Verification items for the finished model (mm, model axes). Face numbers are marked on the shaded views. A direction names the side the tool comes from. Coordinates: 2 decimals unless noted, no trailing zeros. Order: outer loops, then holes, each group sorted by start corner. A loop starts at its lowest first (then second) coordinate and runs counter-clockwise, first axis right, second up. Notation, with made-up numbers: M 46,51.25 L 94,51.25 A21 cw 94,79.25 Z; hole C -4.5,40.25 d3. An arc over 180 degrees is marked long. Return JSON: item names as keys, results as strings. Group by question number.
Q1. Go/stop test with flat-tipped pins: pin 1 Ø5.5 at (x, y) = (-2.5, 38) entering from +Z; pin 2 Ø5.5 at (x, y) = (0, 16) entering from -Z (3 decimals); pin 3 Ø5.5 at (x, y) = (1.5, 18) entering from +Z; pin 4 Ø1 at (x, y) = (-1.5, 4.5) entering from -Z. Record where each tip stops, or that it passes through.
Q2. Section check B-B, the plane z = 17. Enter the section's corners in (x, y).
Q3. Section check D-D, the plane y = -0.5. Enter the section's corners in (x, z), then the cut area to 3 significant figures.
Q4. Section check A-A, the plane y = 36. Enter the section's corners in (x, z), then the cut area to 3 significant figures.
Q5. Thickness scan on probe 1 along Y at (x, z) = (0, -14); probe 2 along Y at (x, z) = (0, -20); probe 3 along Z at (x, y) = (0, -3.25). Record the ranges inside material, lowest first.
Q6. Access from +Z, -Z, +X, -X, +Y, -Y to the whole of each face (thin tool, end or side, straight path). Record for the marked faces 1, 2 and 3.
Q7. Section check C-C, the plane x = 0. Enter the section's corners in (y, z), then the cut area to 3 significant figures.
Q8. Mould release check, pull along Y, two halves, no side actions. Record for the marked faces 4, 5, 6 and 7: pulls with the +Y half, pulls with the -Y half, needs draft (parallel to the pull), parting line crosses it, or undercut.
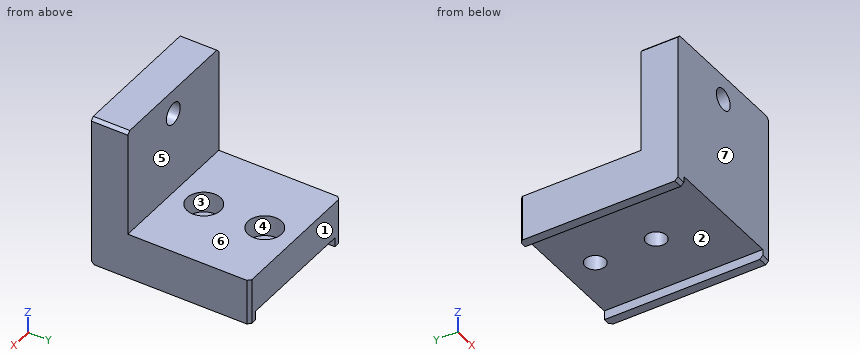
from build123d import *

# Parameters (mm, degrees)
SKETCH_1_W                = 46
SKETCH_1_H                = 50
EXTRUDE_1_DEPTH           = 6
SKETCH_2_W                = 46
SKETCH_2_H                = 15
EXTRUDE_2_DEPTH           = 40
SKETCH_3_W                = 40
SKETCH_3_H                = 52
CUT_EXTRUDE_1_DEPTH       = 3
CHAMFER_1_SIZE            = 1
HOLE_WIZARD_1_D           = 6.6
HOLE_WIZARD_1_CBORE_D     = 11
HOLE_WIZARD_1_CBORE_DEPTH = 6.8
M8X1_0_1_D                = 7


with BuildPart() as part:
    # 草图1 → 凸台-拉伸1 (new, symmetric)
    with BuildSketch(Plane(origin=(0, 0, 0), x_dir=(1, 0, 0), z_dir=(0, 1, 0))):
        Rectangle(SKETCH_1_W, SKETCH_1_H)
    extrude(amount=EXTRUDE_1_DEPTH, both=True)

    # 草图2 → 凸台-拉伸2 (add)
    with BuildSketch(Plane(origin=(0, 6, 0), x_dir=(1, 0, 0), z_dir=(0, 1, 0))):
        with Locations((0, 17.5)):
            Rectangle(SKETCH_2_W, SKETCH_2_H)
    extrude(amount=EXTRUDE_2_DEPTH)

    # 草图3 → 切除-拉伸1 (cut)
    with BuildSketch(Plane(origin=(0, 0, -25), x_dir=(-1, 0, 0), z_dir=(0, 0, -1))):
        with Locations((0, 20)):
            Rectangle(SKETCH_3_W, SKETCH_3_H)
    extrude(amount=-CUT_EXTRUDE_1_DEPTH, mode=Mode.SUBTRACT)

    # 倒角1
    chamfer_1_edges = [part.edges().sort_by_distance(p)[0] for p in [
        (23, 46, -17.5),
        (-23, 46, -17.5),
        (-21.5, -6, -25),
        (21.5, -6, -25),
        (23, 0, 25),
        (-23, 0, 25),
    ]]
    chamfer(chamfer_1_edges, length=CHAMFER_1_SIZE)

    # 打孔尺寸(%根据)内六角圆柱头螺钉的类型1 (through all)
    with Locations(Plane.XY.offset(-10)):
        with Locations((0, 16), (0, 36)):
            CounterBoreHole(HOLE_WIZARD_1_D / 2, HOLE_WIZARD_1_CBORE_D / 2, HOLE_WIZARD_1_CBORE_DEPTH)

    # M8x1.0 螺纹孔1 (through all)
    with Locations(Plane(origin=(0, 6, 0), x_dir=(1, 0, 0), z_dir=(0, 1, 0))):
        with Locations((0, -17)):
            Hole(M8X1_0_1_D / 2)


solid = part.part
Numbers:
{
 "1": {"pin 1": "stops at z = -10", "pin 2": "passes through", "pin 3": "stops at z = -16.8", "pin 4": "stops at z = -22"},
 "2": {"outline": "M -23,-6 L -3.5,-6 L -3.5,6 L -23,6 Z; M 3.5,-6 L 23,-6 L 23,6 L 3.5,6 Z"},
 "3": {"outline": "M -23,-25 L -20,-25 L -20,-22 L 20,-22 L 20,-25 L 23,-25 L 23,24 L 22,25 L -22,25 L -23,24 Z; hole C 0,17 d7", "area": "2,140 mm2"},
 "4": {"outline": "M -23,-25 L -20,-25 L -20,-22 L -3.3,-22 L -3.3,-16.8 L -5.5,-16.8 L -5.5,-10 L -23,-10 Z; M 3.3,-22 L 20,-22 L 20,-25 L 23,-25 L 23,-10 L 5.5,-10 L 5.5,-16.8 L 3.3,-16.8 Z", "area": "461 mm2"},
 "5": {"probe 1": "y = -6 to 10.5, 21.5 to 30.5, 41.5 to 46", "probe 2": "y = -6 to 12.7, 19.3 to 32.7, 39.3 to 46", "probe 3": "z = -22 to 13.5, 20.5 to 25"},
 "6": {"face 1": "+Z, -Z, +X, -X, +Y", "face 2": "-Z, +Y, -Y", "face 3": "+Z"},
 "7": {"outline": "M -6,-22 L 12.7,-22 L 12.7,-16.8 L 10.5,-16.8 L 10.5,-10 L 6,-10 L 6,13.5 L -6,13.5 Z; M -6,20.5 L 6,20.5 L 6,25 L -6,25 Z; M 19.3,-22 L 32.7,-22 L 32.7,-16.8 L 30.5,-16.8 L 30.5,-10 L 21.5,-10 L 21.5,-16.8 L 19.3,-16.8 Z; M 39.3,-22 L 46,-22 L 46,-10 L 41.5,-10 L 41.5,-16.8 L 39.3,-16.8 Z", "area": "742 mm2"},
 "8": {"face 4": "undercut", "face 5": "pulls with the +Y half", "face 6": "needs draft", "face 7": "pulls with the -Y half"}
}
